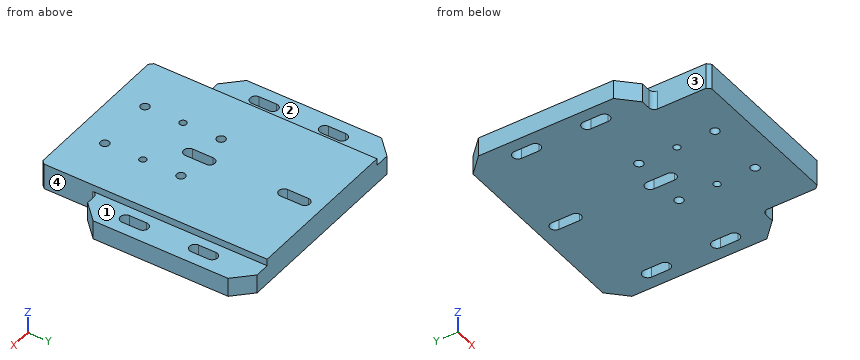
from build123d import *

# Parameters (mm, degrees)
SKETCH1_W               = 130
SKETCH1_H               = 131
EXTRUDE1_DEPTH          = 15
M6_TAPPED_HOLE1_D       = 5
EXTRUDE2_DEPTH          = 94.489304201
SKETCH5_W               = 18.5
SKETCH5_H               = 131
EXTRUDE3_DEPTH          = 4
CHAMFER1_SIZE           = 10
F_4_0_MM_DOWEL_HOLES1_D = 4
EXTRUDE4_DEPTH          = 94.489304201
EXTRUDE5_DEPTH          = 94.489304201
CHAMFER2_SIZE           = 10
CHAMFER3_SIZE           = 2


with BuildPart() as part:
    # Sketch1 → Extrude1 (new body)
    with BuildSketch(Plane.XY):
        Rectangle(SKETCH1_W, SKETCH1_H)
    extrude(amount=EXTRUDE1_DEPTH)

    # M6 Tapped Hole1 (through all)
    with Locations(Plane.XY.offset(15)):
        with Locations((17, -48.5), (-17, -48.5), (-17, -4.5), (17, -4.5)):
            Hole(M6_TAPPED_HOLE1_D / 2)

    # Sketch4 → Extrude2 (cut, through all)
    with BuildSketch(Plane.XY.offset(15)):
        with BuildLine():
            Line((-58.1, -10.5), (-58.1, -0.5))
            ThreePointArc((-58.1, -0.5), (-55, 2.6), (-51.9, -0.5))
            Line((-51.9, -0.5), (-51.9, -10.5))
            ThreePointArc((-51.9, -10.5), (-55, -13.6), (-58.1, -10.5))
        make_face()
        with BuildLine():
            Line((-58.1, 29.5), (-58.1, 39.5))
            ThreePointArc((-58.1, 39.5), (-55, 42.6), (-51.9, 39.5))
            Line((-51.9, 39.5), (-51.9, 29.5))
            ThreePointArc((-51.9, 29.5), (-55, 26.4), (-58.1, 29.5))
        make_face()
        with BuildLine():
            Line((51.9, -10.5), (51.9, -0.5))
            ThreePointArc((51.9, -0.5), (55, 2.6), (58.1, -0.5))
            Line((58.1, -0.5), (58.1, -10.5))
            ThreePointArc((58.1, -10.5), (55, -13.6), (51.9, -10.5))
        make_face()
        with BuildLine():
            Line((51.9, 29.5), (51.9, 39.5))
            ThreePointArc((51.9, 39.5), (55, 42.6), (58.1, 39.5))
            Line((58.1, 39.5), (58.1, 29.5))
            ThreePointArc((58.1, 29.5), (55, 26.4), (51.9, 29.5))
        make_face()
    extrude(amount=-EXTRUDE2_DEPTH, mode=Mode.SUBTRACT)

    # Sketch5 → Extrude3 (cut)
    with BuildSketch(Plane.XY.offset(15)):
        with Locations((-55.75, 0)):
            Rectangle(SKETCH5_W, SKETCH5_H)
        with Locations((55.75, 0)):
            Rectangle(SKETCH5_W, SKETCH5_H)
    extrude(amount=-EXTRUDE3_DEPTH, mode=Mode.SUBTRACT)

    # Chamfer1
    chamfer1_edges = [part.edges().sort_by_distance(p)[0] for p in [
        (-65, 65.5, 5.5),
        (65, 65.5, 5.5),
    ]]
    chamfer(chamfer1_edges, length=CHAMFER1_SIZE)

    # Ø4.0 mm Dowel Holes1 (through all)
    with Locations(Plane(origin=(0, 0, 0), x_dir=(-1, 0, 0), z_dir=(0, 0, -1))):
        with Locations((-17, -26.5), (17, -26.5)):
            Hole(F_4_0_MM_DOWEL_HOLES1_D / 2)

    # Sketch8 → Extrude4 (cut, through all)
    with BuildSketch(Plane.XY.offset(15)):
        with BuildLine():
            Line((-3, 43.5), (-3, 55.5))
            ThreePointArc((-3, 55.5), (0, 58.5), (3, 55.5))
            Line((3, 55.5), (3, 43.5))
            ThreePointArc((3, 43.5), (0, 40.5), (-3, 43.5))
        make_face()
        with BuildLine():
            Line((3, 0.5), (3, -11.5))
            ThreePointArc((3, -11.5), (0, -14.5), (-3, -11.5))
            Line((-3, -11.5), (-3, 0.5))
            ThreePointArc((-3, 0.5), (0, 3.5), (3, 0.5))
        make_face()
    extrude(amount=-EXTRUDE4_DEPTH, mode=Mode.SUBTRACT)

    # Sketch9 → Extrude5 (cut, through all)
    with BuildSketch(Plane.XY.offset(15)):
        with BuildLine():
            Line((-46.5, -65.5), (-65, -65.5))
            Line((-65, -65.5), (-65, -32.5))
            Line((-65, -32.5), (-49.5, -32.5))
            ThreePointArc((-49.5, -32.5), (-47.378679656, -33.378679656), (-46.5, -35.5))
            Line((-46.5, -35.5), (-46.5, -65.5))
        make_face()
        with BuildLine():
            Line((46.5, -65.5), (65, -65.5))
            Line((65, -65.5), (65, -32.5))
            Line((65, -32.5), (49.5, -32.5))
            ThreePointArc((49.5, -32.5), (47.378679656, -33.378679656), (46.5, -35.5))
            Line((46.5, -35.5), (46.5, -65.5))
        make_face()
    extrude(amount=-EXTRUDE5_DEPTH, mode=Mode.SUBTRACT)

    # Chamfer2
    chamfer2_edges = [part.edges().sort_by_distance(p)[0] for p in [
        (-65, -32.5, 5.5),
        (65, -32.5, 5.5),
    ]]
    chamfer(chamfer2_edges, length=CHAMFER2_SIZE)

    # Chamfer3
    chamfer3_edges = [part.edges().sort_by_distance(p)[0] for p in [
        (-46.5, -65.5, 7.5),
        (46.5, -65.5, 7.5),
    ]]
    chamfer(chamfer3_edges, length=CHAMFER3_SIZE)


solid = part.part
Build history of the part. All positions in model axes, mm. Face numbers are marked on the shaded views. A direction names the side the tool comes from. Coordinates: 2 decimals unless noted, no trailing zeros. Order: outer loops, then holes, each group sorted by start corner. A loop starts at its lowest first (then second) coordinate and runs counter-clockwise, first axis right, second up. Notation, with made-up numbers: (-32.75, 35) - (0.25, 35) arc R25 cw to (0.25, 64) - close; hole circle Ø5 at (80.25, 87.25). An arc over 180 degrees is marked (long way). Write each question's results on one line, items separated by ' | '. Start each with the question number.
Item 1: Band-saw the part on B-B on y = -26.5. Write the cut outline in (x, z).
Item 2: Band-saw the part on D-D on z = 8.25. State how many separate pieces and enclosed holes the cut face has, and give its area (3 significant figures).
Item 3: Band-saw the part on C-C on y = 16. Write the cut outline in (x, z).
Item 4: Flat gauge pins, fed straight in: pin 1 (9 mm diameter, centred on x = 57.5, y = 12, fed in from +Z); pin 2 (4.5 mm diameter, centred on x = -52.5, z = 5, fed in from -Y); pin 3 (4 mm diameter, centred on x = -17, y = -4.5, fed in from -Z). Where does each tip first touch, or does it go through?
Item 5: Wall check: probe 1 along Y at (x, z) = (17, 9.25); probe 2 along X at (y, z) = (-10, 2.5); probe 3 along Y at (x, z) = (-51, 0.75). Give the ranges that are in metal, low to high. Write a range as [from, to].
Item 6: Tool access for the marked faces 1, 2, 3 and 4: list every direction of +Z, -Z, +X, -X, +Y, -Y with a clear straight run to the whole face (end or side of a thin tool).
Item 7: Band-saw the part on A-A on x = 17. Write the cut outline in (y, z).
Numbers:
1) outline: (-61, 0) - (-19, 0) - (-19, 15) - (-46.5, 15) - (-46.5, 11) - (-61, 11) - close; (-15, 0) - (15, 0) - (15, 15) - (-15, 15) - close; (19, 0) - (61, 0) - (61, 11) - (46.5, 11) - (46.5, 15) - (19, 15) - close
2) separate pieces: 1 | enclosed holes: 12 | area: 14,900 mm^2
3) outline: (-65, 0) - (65, 0) - (65, 11) - (46.5, 11) - (46.5, 15) - (-46.5, 15) - (-46.5, 11) - (-65, 11) - close
4) pin 1: z = 11 | pin 2: y = -32.5 | pin 3: through
5) probe 1: [-65.5, -51], [-46, -28.5], [-24.5, -7], [-2, 65.5] | probe 2: [-65, -58.1], [-51.9, -3], [3, 51.9], [58.1, 65] | probe 3: [-32.5, 65.5]
6) face 1: +Z, +X, +Y, -Y | face 2: +Z, -X, +Y, -Y | face 3: +Z, -X, -Y | face 4: +Z, +X, -Y
7) outline: (-65.5, 0) - (-51, 0) - (-51, 15) - (-65.5, 15) - close; (-46, 0) - (-28.5, 0) - (-28.5, 15) - (-46, 15) - close; (-24.5, 0) - (-7, 0) - (-7, 15) - (-24.5, 15) - close; (-2, 0) - (65.5, 0) - (65.5, 15) - (-2, 15) - close
